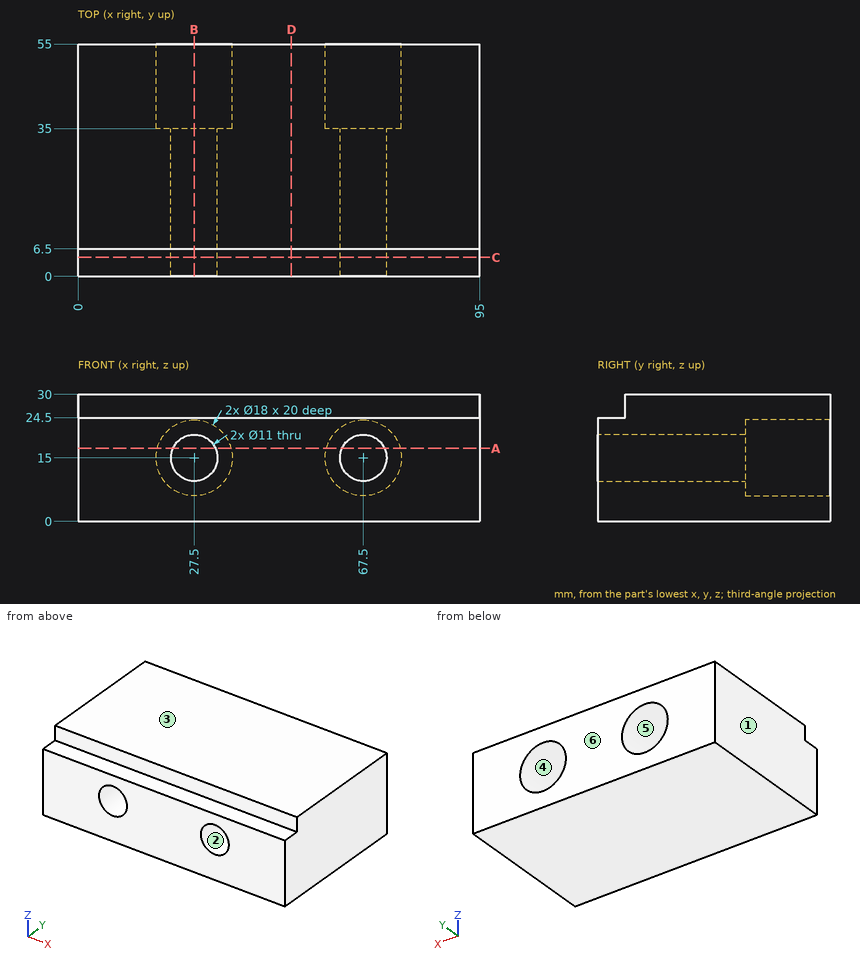
Study the drawing (mm; zero at the part's minimum x, y, z) and answer. A direction names the side the tool comes from. Give positions to 0.01 mm unless a question says otherwise; leave off trailing zeros. Order: outer loops, then holes, each group sorted by start corner. A loop starts at its lowest first (then second) coordinate and runs counter-clockwise, first axis right, second up. Notation, with made-up numbers: (-39, 80) - (11, 80) arc R15 ccw to (11, 100) - close; hole circle Ø4 at (54.5, 15.5). An arc over 180 degrees is marked (long way). Answer as CSV lines item,"result". Start each with the question number.
Q1. Find the intervals of material crossed by L1, parallel to X at y = 8, z = 15; L2, parallel to X at y = 7, z = 14; L3, parallel to Z at x = 67, y = 25, in increasing order. Write a range as [from, to].
Q2. The part is cut by section D-D (x = 50.5). Write down the section's boundary in (y, z), then the cut area to 3 significant figures.
Q3. The part is cut by section A-A (z = 17.25). Write down the section's boundary in (x, y), then the cut area to 3 significant figures.
Q4. The part is cut by section B-B (x = 27.5). Write down the section's boundary in (y, z).
Q5. The mould has two halves that part along X. Classify the marked faces 1, 2, 3 and 4: +X half, -X half, draft (parallel to the pull), parting line (faces both ways), or undercut.
Q6. For the marked faces 5 and 6, determine the directions among +Z, -Z, +X, -X, +Y, -Y from which every point of the face is accessible in a straight line to the end or side of a thin tool.
Q7. The part is cut by section C-C (y = 4.5). Write down the section's boundary in (x, z), then the cut area to 3 significant figures.
Q8. Given pin 1 Ø3 at (x, y) = (55.5, 2) entering from +Z; pin 2 Ø9 at (x, z) = (25, 18) entering from +Y; pin 3 Ø9 at (x, z) = (67.5, 15) entering from +Y; pin 4 Ø3 at (x, z) = (31.5, 27.5) entering from -Y, each flat-ended and moving along its own axis, determine where each tip first touches the part or whether it passes through.
Check result:
1,L1,"x = [0, 22], [33, 62], [73, 95]"
1,L2,"x = [0, 22.09], [32.91, 62.09], [72.91, 95]"
1,L3,"z = [0, 9.52], [20.48, 30]"
2,outline,"(0, 0) - (55, 0) - (55, 30) - (6.5, 30) - (6.5, 24.5) - (0, 24.5) - close"
2,area,"1,610 mm²"
3,outline,"(0, 0) - (22.48, 0) - (22.48, 35) - (18.79, 35) - (18.79, 55) - (0, 55) - close; (32.52, 0) - (62.48, 0) - (62.48, 35) - (58.79, 35) - (58.79, 55) - (36.21, 55) - (36.21, 35) - (32.52, 35) - close; (72.52, 0) - (95, 0) - (95, 55) - (76.21, 55) - (76.21, 35) - (72.52, 35) - close"
3,area,"3,830 mm²"
4,outline,"(0, 0) - (55, 0) - (55, 6) - (35, 6) - (35, 9.5) - (0, 9.5) - close; (0, 20.5) - (35, 20.5) - (35, 24) - (55, 24) - (55, 30) - (6.5, 30) - (6.5, 24.5) - (0, 24.5) - close"
5,face 1,"-X half"
5,face 2,"undercut"
5,face 3,"draft"
5,face 4,"undercut"
6,face 5,"+Y"
6,face 6,"+Z, -Z, +X, -X, +Y"
7,outline,"(0, 0) - (95, 0) - (95, 24.5) - (0, 24.5) - close; hole circle Ø11 at (27.5, 15); hole circle Ø11 at (67.5, 15)"
7,area,"2,140 mm²"
8,pin 1,"stops at z = 24.5"
8,pin 2,"stops at y = 35"
8,pin 3,"passes through"
8,pin 4,"stops at y = 6.5"
